Design review of the part built by this model. Coordinates are the model's own, in mm. A direction names the side the tool comes from. Coordinates: 2 decimals unless noted, no trailing zeros. Write each loop counter-clockwise with the first axis right and the second up, starting at its lowest first coordinate (ties: lowest second). Pieces come first, ordered by that corner, then holes. Notation, with made-up numbers: (5, -12) - (50, -12) arc R25 cw to (50, 11) - close; hole circle Ø9 at (5, 26). An arc over 180 degrees is marked (long way). Use a Markdown table: item, result.
from build123d import *

# Parameters (mm, degrees)
BRACKET_BODY_DEPTH        = 82
BODY_CORNER_FILLETS_R12_R = 12
MOUNTING_HOLES_SKETCH_R   = 5
MOUNTING_HOLES_DEPTH      = 152.19523802
CENTRE_RIB_12MM_REACH     = 135.48
RIB_SKETCH_WALL_W         = 368.920663258
RIB_SKETCH_WALL_H         = 12
INNER_CORNER_FILLET_R12_R = 12
CRADLE_BOSS_DEPTH         = 30


with BuildPart() as part:
    # Bracket Profile Sketch → Bracket Body (new body)
    with BuildSketch(Plane(origin=(0, 0, 0), x_dir=(0, 0, -1), z_dir=(1, 0, 0))):
        Polygon((0, 0), (12, 0), (12, 24), (94, 24), (94, 0), (106, 0), (106, 70), (94, 70), (94, 36), (0, 36), align=None)
    extrude(amount=BRACKET_BODY_DEPTH)

    # Body Corner Fillets R12
    body_corner_fillets_r12_edges = [part.edges().sort_by_distance(p)[0] for p in [
        (0, 0, -100),
        (0, 0, -6),
        (82, 0, -100),
        (82, 0, -6),
    ]]
    fillet(body_corner_fillets_r12_edges, radius=BODY_CORNER_FILLETS_R12_R)

    # Mounting Holes Sketch → Mounting Holes (cut, through all)
    with BuildSketch(Plane.XY):
        with Locations((12, 12)):
            Circle(MOUNTING_HOLES_SKETCH_R)
        with Locations((70, 12)):
            Circle(MOUNTING_HOLES_SKETCH_R)
    extrude(amount=-MOUNTING_HOLES_DEPTH, mode=Mode.SUBTRACT)

    # Rib Sketch wall → Centre Rib 12mm (add, up to next)
    with BuildSketch(Plane(origin=(41, 53, -47), x_dir=(0, -0.340136081654, 0.940376225751), z_dir=(0, -0.940376225751, -0.340136081654)), mode=Mode.PRIVATE) as centre_rib_12mm_sk1:
        Rectangle(RIB_SKETCH_WALL_W, RIB_SKETCH_WALL_H)
    centre_rib_12mm_tool1 = extrude(centre_rib_12mm_sk1.sketch, amount=CENTRE_RIB_12MM_REACH, mode=Mode.PRIVATE) - part.part
    add(centre_rib_12mm_tool1.solids().sort_by_distance((41, 53, -47))[0])

    # Inner Corner Fillet R12
    inner_corner_fillet_r12_edges = [part.edges().sort_by_distance(p)[0] for p in [
        (64.5, 36, -94),
        (17.5, 36, -94),
    ]]
    fillet(inner_corner_fillet_r12_edges, radius=INNER_CORNER_FILLET_R12_R)

    # Cradle Profile Sketch → Cradle Boss (add, symmetric)
    with BuildSketch(Plane(origin=(41, 0, 0), x_dir=(0, 0, -1), z_dir=(1, 0, 0))):
        with BuildLine():
            Line((120.994884686, 70), (137.998837993, 70))
            ThreePointArc((137.998837993, 70), (132.322243398, 55.475371387), (118.444444444, 48.362336959))
            ThreePointArc((118.444444444, 48.362336959), (109.565016105, 43.782358433), (106, 34.449025099))
            Line((106, 34.449025099), (106, 70))
            Line((106, 70), (111.005115314, 70))
            ThreePointArc((111.005115314, 70), (116, 65.226112739), (120.994884686, 70))
        make_face()
    extrude(amount=CRADLE_BOSS_DEPTH, both=True)


solid = part.part
(1) For pin 1 (9.5 mm diameter, centred on y = 46, z = -123.5, fed in from +X); pin 2 (8 mm diameter, centred on x = 67, z = -55.5, fed in from +Y); pin 3 (4 mm diameter, centred on x = 25.5, z = -78, fed in from -Y); pin 4 (6 mm diameter, centred on x = 70, y = 12, fed in from -Z), all flat-tipped, find the tip position at first contact; note any pin that passes through.
Determined:
| item | result |
|---|---|
| pin 1 | x = 71 |
| pin 2 | y = 36 |
| pin 3 | y = 24 |
| pin 4 | through |
(2) Machinability: for faces 1 (the flat face through (41, 70, -129)), 2 (the flat face through (17, 36, -42)), 3 (the flat face through (71, 60, -119)), 4 (the cylindrical face through (74.77, 13.5, -5.92)), 5 (the flat face through (40, 12, -12)), which of the approach directions +Z, -Z, +X, -X, +Y, -Y give a long, thin tool a straight path to every point of the face, cutting with its end or side? Answer none if there is none.
Determined:
| item | result |
|---|---|
| face 1 | +Z, -Z, +X, -X, +Y |
| face 2 | +Z, -X, +Y |
| face 3 | -Z, +X, +Y, -Y |
| face 4 | +Z, -Z |
| face 5 | +X, -X, -Y |
(3) Take a section at A-A on z = -99.5. Write out the cut boundary in (x, y), and give its area (3 significant figures).
Determined:
| item | result |
|---|---|
| outline | (0, 12) arc R12 ccw to (12, 0) - (70, 0) arc R12 ccw to (82, 12) - (82, 70) - (0, 70) - close; hole circle Ø10 at (12, 12); hole circle Ø10 at (70, 12) |
| area | 5,520 mm2 |
(4) Take a section at D-D on z = -116. Write out the cut boundary in (x, y).
Determined:
| item | result |
|---|---|
| outline | (11, 47.87) - (71, 47.87) - (71, 65.23) - (11, 65.23) - close |
(5) Take a section at B-B on z = -17.5. Write out the cut boundary in (x, y), and give its area (3 significant figures).
Determined:
| item | result |
|---|---|
| outline | (0, 24) - (82, 24) - (82, 36) - (47, 36) - (47, 42.33) - (35, 42.33) - (35, 36) - (0, 36) - close |
| area | 1,060 mm2 |
(6) Take a section at C-C on z = -66. Write out the cut boundary in (x, y).
Determined:
| item | result |
|---|---|
| outline | (0, 24) - (82, 24) - (82, 36) - (47, 36) - (47, 59.87) - (35, 59.87) - (35, 36) - (0, 36) - close |
(7) For L1, parallel to Z at x = 66, y = 7.5; L2, parallel to Y at x = 12, z = -4.75; L3, parallel to Y at x = 24.5, z = -20, list the stretches that pass through material, from the lowest coordinate up. Write a range as from..to.
Determined:
| item | result |
|---|---|
| L1 | -106..-94, -12..0 |
| L2 | 0..7, 17..36 |
| L3 | 24..36 |
(8) Draft analysis for pull direction Y (two halves, no side actions). For faces 6 (the cylindrical face through (78.39, 3.42, -100.08)), 7 (the flat face through (40, 12, -94)), 8 (the cylindrical face through (16.77, 13.5, -5.92)), state which applies: +Y half, -Y half, draft (parallel to the pull), parting line (faces both ways), or undercut.
Determined:
| item | result |
|---|---|
| face 6 | -Y half |
| face 7 | draft |
| face 8 | undercut |
